Source: three-view drawing plus pictorial views. Frame: mm from the lowest corner of the part. Give positions to 0.01 mm unless a question says otherwise; leave off trailing zeros. Loops run counter-clockwise (first coordinate to the right, second up) from the corner with the lowest first, then second, coordinate; pieces in that order, holes last. Notation, with made-up numbers: M -7,-31 L 46,-31 A9 ccw 46,-27 Z; hole C 4.5,43 d3. An arc over 180 degrees is marked long. Answer as a JSON object with one key per item and string values. Group by question number.
1) Section query A-A on z = 32. Return loops of the section in (x, y).
2) First-contact query: P1, Ø2, axis at x = 339, z = 18.5, coming from the +Y side; P2, Ø6, axis at x = 645, z = 4.5, coming from the -Y side; P3, Ø20, axis at y = 780.5, z = 15, coming from the +X side. Flat tips, straight axial feed; report the tip coordinate or a pass-through.
3) Ray query, L1, parallel to X at y = 401, z = 15; L2, parallel to Y at x = 890, z = 11; L3, parallel to Y at x = 508, z = 20. Return the intervals inside material, ascending.
4) Section query B-B on y = 767. Return loops of the section in (x, z), plus the area to 3 significant figures.
5) Section query C-C on x = 608. Return loops of the section in (y, z), plus the area to 3 significant figures.
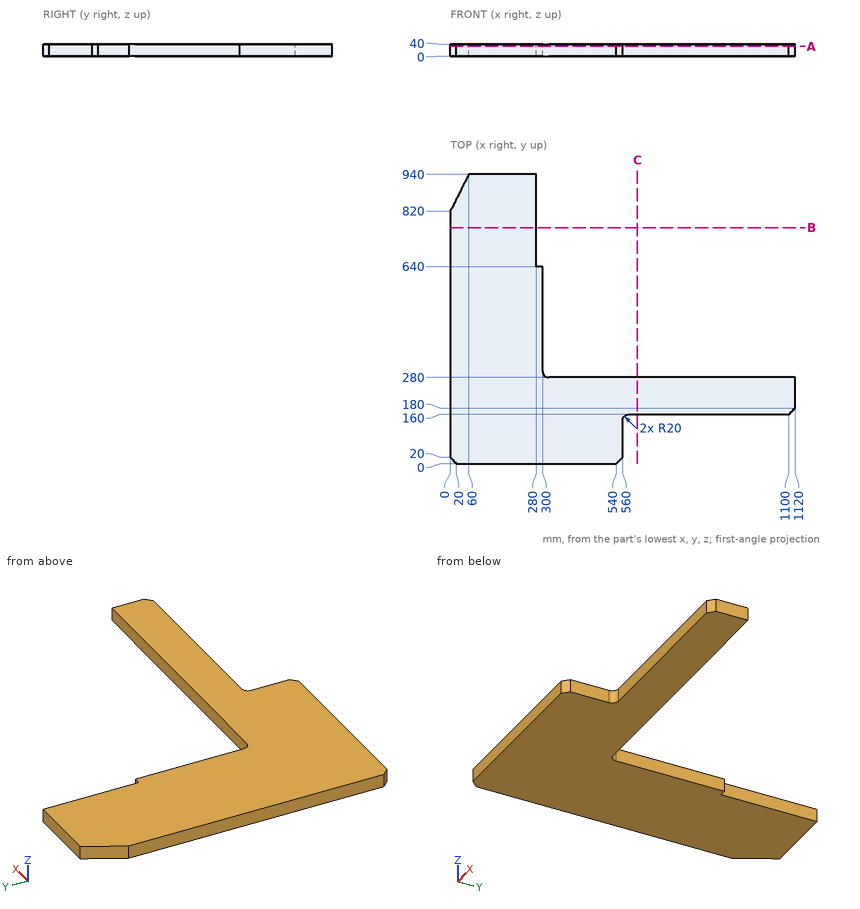
Output:
{
 "1": {"outline": "M 0,20 L 20,0 L 540,0 L 560,20 L 560,140 A20 cw 580,160 L 1100,160 L 1120,180 L 1120,280 L 320,280 A20 cw 300,300 L 300,640 L 280,640 L 280,940 L 60,940 L 0,820 Z"},
 "2": {"P1": "stops at y = 280", "P2": "stops at y = 160", "P3": "stops at x = 280"},
 "3": {"L1": "x = 0 to 300", "L2": "y = 160 to 280", "L3": "y = 0 to 280"},
 "4": {"outline": "M 0,0 L 280,0 L 280,40 L 0,40 Z", "area": "11,200 mm^2"},
 "5": {"outline": "M 160,0 L 280,0 L 280,40 L 160,40 Z", "area": "4,800 mm^2"}
}
